The model under review builds one solid part; all positions refer to its coordinate system, in mm. A direction names the side the tool comes from. Round coordinates to 2 decimals unless told otherwise and drop trailing zeros. Write each loop counter-clockwise with the first axis right and the second up, starting at its lowest first coordinate (ties: lowest second). Pieces come first, ordered by that corner, then holes. Notation, with made-up numbers: (41, 50) - (56, 50) arc R28 cw to (56, 82) - close; hole circle Ø6 at (-36.75, -20). An arc over 180 degrees is marked (long way). Write each question's results on one line, items separated by ' | '.
```python
from build123d import *

# Parameters (mm, degrees)
HEXALOBULAR_REACH = 30.827


with BuildPart() as part:
    # BodySke → Base-Revolve (revolve)
    with BuildSketch(Plane(origin=(0, 0, 0), x_dir=(0, 0, -1), z_dir=(1, 0, 0)), mode=Mode.PRIVATE) as base_revolve_sk:
        with BuildLine():
            Line((3.130026132, 9.15), (7.280026132, 5))
            Line((7.280026132, 5), (26.280026132, 5))
            Line((26.280026132, 5), (26.280026132, 0))
            Line((26.280026132, 0), (0, 0))
            ThreePointArc((0, 0), (0.578590295, 4.714897114), (2.280026132, 9.15))
            Line((2.280026132, 9.15), (3.130026132, 9.15))
        make_face()
    revolve(base_revolve_sk.sketch.rotate(Axis((0, 0, 0), (0, 0, 1)), 90), axis=Axis((0, 0, 0), (0, 0, 1)))

    # PreBSke → PreBroach (revolve, cut)
    with BuildSketch(Plane(origin=(0, 0, 0), x_dir=(0, 0, -1), z_dir=(1, 0, 0))):
        Polygon((0, 0), (0, 4.475), (3.42, 4.475), (6.10885127, 0), align=None)
    revolve(axis=Axis((0, 0, 0), (0, 0, 1)), mode=Mode.SUBTRACT)

    # Hexalobular: up to this cone (the profile starts inside it)
    hexalobular_end = Plane(origin=(0, 0, -0.520422), z_dir=(0, 0, 1)).offset(-5.58842827) * Cone(1.664e-06, 76.9165693, 46.216136443, align=(Align.CENTER, Align.CENTER, Align.MIN), mode=Mode.PRIVATE)
    # HexSke → Hexalobular (add, up to the surface)
    with BuildSketch(Plane.XY.offset(-0.52042216), mode=Mode.PRIVATE) as hexalobular_sk1:
        with BuildLine():
            ThreePointArc((-3.875463682, -2.2375), (-3.985930746, -1.660351093), (-3.714652929, -1.139090909))
            ThreePointArc((-3.714652929, -1.139090909), (-3.2233964, 0), (-3.714652929, 1.139090909))
            ThreePointArc((-3.714652929, 1.139090909), (-3.985930746, 1.660351093), (-3.875463682, 2.2375))
            ThreePointArc((-3.875463682, 2.2375), (-4.475, 0), (-3.875463682, -2.2375))
        make_face()
    hexalobular_tool1 = extrude(hexalobular_sk1.sketch, amount=-HEXALOBULAR_REACH, mode=Mode.PRIVATE) & hexalobular_end
    add(hexalobular_tool1.solids().sort_by_distance((-3.918157, 0, -0.520422))[0])
    # HexSke → Hexalobular (add, up to the surface)
    with BuildSketch(Plane.XY.offset(-0.52042216), mode=Mode.PRIVATE) as hexalobular_sk2:
        with BuildLine():
            ThreePointArc((-2.843808129, -2.647438348), (-3.430871599, -2.621741738), (-3.875463682, -2.2375))
            ThreePointArc((-3.875463682, -2.2375), (-2.2375, -3.875463682), (0, -4.475))
            ThreePointArc((0, -4.475), (-0.555059148, -4.282092831), (-0.8708448, -3.786529257))
            ThreePointArc((-0.8708448, -3.786529257), (-1.6116982, -2.791543169), (-2.843808129, -2.647438348))
        make_face()
    hexalobular_tool2 = extrude(hexalobular_sk2.sketch, amount=-HEXALOBULAR_REACH, mode=Mode.PRIVATE) & hexalobular_end
    add(hexalobular_tool2.solids().sort_by_distance((-1.959079, -3.393224, -0.520422))[0])
    # HexSke → Hexalobular (add, up to the surface)
    with BuildSketch(Plane.XY.offset(-0.52042216), mode=Mode.PRIVATE) as hexalobular_sk3:
        with BuildLine():
            ThreePointArc((0, 4.475), (-2.2375, 3.875463682), (-3.875463682, 2.2375))
            ThreePointArc((-3.875463682, 2.2375), (-3.430871599, 2.621741738), (-2.843808129, 2.647438348))
            ThreePointArc((-2.843808129, 2.647438348), (-1.6116982, 2.791543169), (-0.8708448, 3.786529257))
            ThreePointArc((-0.8708448, 3.786529257), (-0.555059148, 4.282092831), (0, 4.475))
        make_face()
    hexalobular_tool3 = extrude(hexalobular_sk3.sketch, amount=-HEXALOBULAR_REACH, mode=Mode.PRIVATE) & hexalobular_end
    add(hexalobular_tool3.solids().sort_by_distance((-1.959079, 3.393224, -0.520422))[0])
    # HexSke → Hexalobular (add, up to the surface)
    with BuildSketch(Plane.XY.offset(-0.52042216), mode=Mode.PRIVATE) as hexalobular_sk4:
        with BuildLine():
            ThreePointArc((0.8708448, -3.786529257), (0.555059148, -4.282092831), (0, -4.475))
            ThreePointArc((0, -4.475), (2.2375, -3.875463682), (3.875463682, -2.2375))
            ThreePointArc((3.875463682, -2.2375), (3.430871599, -2.621741738), (2.843808129, -2.647438348))
            ThreePointArc((2.843808129, -2.647438348), (1.6116982, -2.791543169), (0.8708448, -3.786529257))
        make_face()
    hexalobular_tool4 = extrude(hexalobular_sk4.sketch, amount=-HEXALOBULAR_REACH, mode=Mode.PRIVATE) & hexalobular_end
    add(hexalobular_tool4.solids().sort_by_distance((1.959079, -3.393224, -0.520422))[0])
    # HexSke → Hexalobular (add, up to the surface)
    with BuildSketch(Plane.XY.offset(-0.52042216), mode=Mode.PRIVATE) as hexalobular_sk5:
        with BuildLine():
            ThreePointArc((3.875463682, 2.2375), (2.2375, 3.875463682), (0, 4.475))
            ThreePointArc((0, 4.475), (0.555059148, 4.282092831), (0.8708448, 3.786529257))
            ThreePointArc((0.8708448, 3.786529257), (1.6116982, 2.791543169), (2.843808129, 2.647438348))
            ThreePointArc((2.843808129, 2.647438348), (3.430871599, 2.621741738), (3.875463682, 2.2375))
        make_face()
    hexalobular_tool5 = extrude(hexalobular_sk5.sketch, amount=-HEXALOBULAR_REACH, mode=Mode.PRIVATE) & hexalobular_end
    add(hexalobular_tool5.solids().sort_by_distance((1.959079, 3.393224, -0.520422))[0])
    # HexSke → Hexalobular (add, up to the surface)
    with BuildSketch(Plane.XY.offset(-0.52042216), mode=Mode.PRIVATE) as hexalobular_sk6:
        with BuildLine():
            ThreePointArc((3.714652929, -1.139090909), (3.985930746, -1.660351093), (3.875463682, -2.2375))
            ThreePointArc((3.875463682, -2.2375), (4.475, 0), (3.875463682, 2.2375))
            ThreePointArc((3.875463682, 2.2375), (3.985930746, 1.660351093), (3.714652929, 1.139090909))
            ThreePointArc((3.714652929, 1.139090909), (3.2233964, 0), (3.714652929, -1.139090909))
        make_face()
    hexalobular_tool6 = extrude(hexalobular_sk6.sketch, amount=-HEXALOBULAR_REACH, mode=Mode.PRIVATE) & hexalobular_end
    add(hexalobular_tool6.solids().sort_by_distance((3.918157, 0, -0.520422))[0])

    # ThdSchSke → ThreadSchematic (revolve, cut)
    with BuildSketch(Plane(origin=(0, 0, 0), x_dir=(0, 0, -1), z_dir=(1, 0, 0))):
        Polygon((26.758072155, 5), (26.280026132, 4.172), (25.80198011, 5), align=None)
    revolve(axis=Axis((0, 0, 0), (0, 0, 1)), mode=Mode.SUBTRACT)


solid = part.part
```
Q1. The part is to be moulded in two halves that separate along X. For faces 4 (the cylindrical face through (1.6, -2.8, -2.3)), 5 (the conical face through (4.128, 3.165, -7.079)), 6 (the flat face through (-4, 0, -0.52)), 7 (the cylindrical face through (3.223, 0.018, -2.321)), say which applies: released by +X, released by -X, zero draft, split by the parting line, or undercut.
Evaluation:
face 4: undercut | face 5: split by the parting line | face 6: zero draft | face 7: undercut
Q2. We need section B-B (z = -20.75). State the section outline as (x, y) points, plus the area to 3 significant figures.
Evaluation:
outline: circle Ø10 at (0, 0) | area: 78.5 mm^2
Q3. Insertion check: P1, Ø4, axis at x = 7, y = 7.5, coming from the -Z side; P2, Ø5, axis at y = -1.5, z = -22, coming from the +X side; P3, Ø2, axis at x = -0.5, z = -4.5, coming from the -Y side. Each pin has a flat end and moves straight along its axis. Give the tip position at first contact, or say it passes through.
Evaluation:
P1: stops at z = -4.02 | P2: stops at x = 5 | P3: stops at y = -8.77
Q4. For probe 1 along X at (y, z) = (1, -4); probe 2 along Y at (x, z) = (-2.25, -2.75); probe 3 along Y at (x, z) = (0.75, -2), list the stretches that pass through material, from the lowest coordinate up.
Evaluation:
probe 1: x = -8.22 to -3.36, 3.36 to 8.22 | probe 2: y = -8.87 to -2.59, 2.59 to 8.87 | probe 3: y = -8.57 to -4.07, 4.07 to 8.57
Q5. We need section A-A (z = -4.5). State the section outline as (x, y) points, plus the area to 3 significant figures.
Evaluation:
outline: circle Ø15.56 at (0, 0); hole circle Ø5.36 at (0, 0) | area: 168 mm^2
Q6. Tool access review of faces 1 (the cylindrical face through (-4.77, -1.5, -16.67)), 2 (the flat face through (2, -3, -0.52)), 3 (the cylindrical face through (-1.6, -2.8, -2.3)): name each direction out of +Z, -Z, +X, -X, +Y, -Y from which nothing blocks a thin tool from reaching the whole face with its end or side.
Evaluation:
face 1: -Z | face 2: +Z, +X, -X, +Y, -Y | face 3: +Z
